from build123d import *

# Parameters (mm, degrees)
EXTRUDE_406_DEPTH   = 240
SKETCH_3_R          = 2.5
SKETCH_3_R_2        = 3
CUT_EXTRUDE_1_DEPTH = 10


with BuildPart() as part:
    # 草图1 → Extrude 406 (new body)
    with BuildSketch(Plane.XY):
        with BuildLine():
            Line((33, 50.785428571), (15, 50.785428571))
            Line((15, 50.785428571), (15, 50.285428571))
            Line((15, 50.285428571), (-15, 50.285428571))
            Line((-15, 50.285428571), (-15, 50.785428571))
            Line((-15, 50.785428571), (-33, 50.785428571))
            ThreePointArc((-33, 50.785428571), (-36.535533906, 49.320962477), (-38, 45.785428571))
            Line((-38, 45.785428571), (-38, 9.785428571))
            ThreePointArc((-38, 9.785428571), (-37.121320344, 7.664108228), (-35, 6.785428571))
            Line((-35, 6.785428571), (-25, 6.785428571))
            Line((-25, 6.785428571), (-25, 39.785428571))
            Line((-25, 39.785428571), (25, 39.785428571))
            Line((25, 39.785428571), (25, 6.785428571))
            Line((25, 6.785428571), (35, 6.785428571))
            ThreePointArc((35, 6.785428571), (37.121320344, 7.664108228), (38, 9.785428571))
            Line((38, 9.785428571), (38, 45.785428571))
            ThreePointArc((38, 45.785428571), (36.535533906, 49.320962477), (33, 50.785428571))
        make_face()
    extrude(amount=-EXTRUDE_406_DEPTH)

    # 草图3 → 切除-拉伸1 (cut)
    with BuildSketch(Plane(origin=(0, 50.785428571, 0), x_dir=(-1, 0, 0), z_dir=(0, 1, 0))):
        with Locations((-20, -24)):
            Circle(SKETCH_3_R)
        with Locations((20, -24)):
            Circle(SKETCH_3_R)
        with Locations((-20, -88)):
            Circle(SKETCH_3_R)
        with Locations((20, -88)):
            Circle(SKETCH_3_R)
        with Locations((-20, -152)):
            Circle(SKETCH_3_R)
        with Locations((20, -152)):
            Circle(SKETCH_3_R)
        with Locations((-20, -216)):
            Circle(SKETCH_3_R)
        with Locations((20, -216)):
            Circle(SKETCH_3_R)
        with Locations((-25, -73)):
            Circle(SKETCH_3_R_2)
        with Locations((25, -73)):
            Circle(SKETCH_3_R_2)
        with Locations((-25, -167)):
            Circle(SKETCH_3_R_2)
        with Locations((25, -167)):
            Circle(SKETCH_3_R_2)
    extrude(amount=-CUT_EXTRUDE_1_DEPTH, mode=Mode.SUBTRACT)


solid = part.part
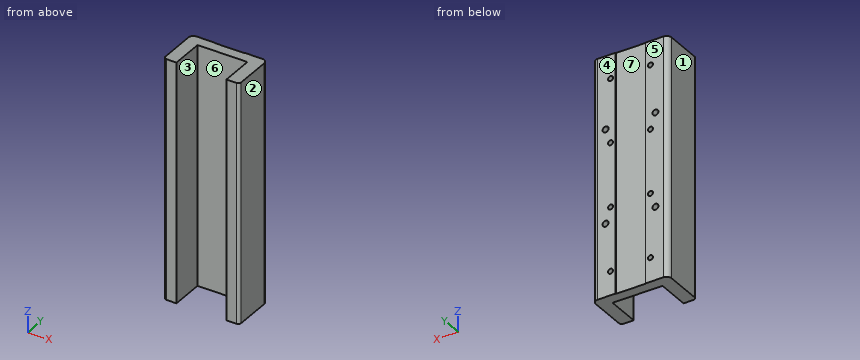
Part model, mm, in its own coordinate system. Face numbers are marked on the shaded views. A direction names the side the tool comes from. Coordinates: 2 decimals unless noted, no trailing zeros. Loops run counter-clockwise (first coordinate to the right, second up) from the corner with the lowest first, then second, coordinate; pieces in that order, holes last. Notation, with made-up numbers: (31.5, -34) - (76.5, -34) arc R15 ccw to (76.5, -23) - close; hole circle Ø3 at (3.5, 33). An arc over 180 degrees is marked (long way). Write each question's results on one line, items separated by ' | '. Start each with the question number.
Q1. Slice it at B-B on z = -73. Give the cut face in (x, y), and give its area (3 significant figures).
Q2. Which spindle directions (+Z, -Z, +X, -X, +Y, -Y) get a long thin tool onto all of the face, cutting with end or side? Do the marked faces 5, 6 and 7. Say none if no direction does.
Q3. Slice it at A-A on y = 31. Give the cut face in (x, z), and give its area (3 significant figures).
Q4. Probe line 1 along Z through (x, y) = (25, 45); line 2 along Z through (x, y) = (20, 47); line 3 along X through (y, z) = (45, -152). List the from-to ranges inside material, lowest first.
Q5. Drop flat-ended pins along their axis: pin 1 Ø1.8 at (x, z) = (-25.5, -167) entering from +Y; pin 2 Ø6.5 at (x, z) = (-20, -24) entering from +Y; pin 3 Ø12 at (x, z) = (13.5, -208) entering from -Y. Give the stop position or say it passes through.
Q6. Slice it at D-D on x = 7.5. Give the cut face in (y, z), and give its area (3 significant figures).
Q7. Slice it at C-C on y = 48. Give the number of separate pieces and of enclosed holes in the cut face, and give its area (3 significant figures).
Q8. Two-plate mould, pull along X, no slides. Class the marked faces 1, 2, 3 and 4: +X half, -X half, draft (parallel to the pull), parting line (faces both ways), or undercut.
Answer:
1) outline: (-38, 9.79) arc R3 ccw to (-35, 6.79) - (-25, 6.79) - (-25, 39.79) - (25, 39.79) - (25, 6.79) - (35, 6.79) arc R3 ccw to (38, 9.79) - (38, 45.79) arc R5 ccw to (33, 50.79) - (28, 50.79) - (28, 40.79) - (22, 40.79) - (22, 50.79) - (15, 50.79) - (15, 50.29) - (-15, 50.29) - (-15, 50.79) - (-22, 50.79) - (-22, 40.79) - (-28, 40.79) - (-28, 50.79) - (-33, 50.79) arc R5 ccw to (-38, 45.79) - close | area: 1,540 mm2
2) face 5: +Z, -Z, +X, -X, +Y | face 6: +Z, -Z, -Y | face 7: +Z, -Z, +Y
3) outline: (-38, -240) - (-25, -240) - (-25, 0) - (-38, 0) - close; (25, -240) - (38, -240) - (38, 0) - (25, 0) - close | area: 6,240 mm2
4) line 1: z = -240 to -170, -164 to -76, -70 to 0 | line 2: z = -240 to -218.5, -213.5 to -154.5, -149.5 to -90.5, -85.5 to -26.5, -21.5 to 0 | line 3: x = -38 to -22.5, -17.5 to 17.5, 22.5 to 38
5) pin 1: stops at y = 40.79 | pin 2: stops at y = 50.79 | pin 3: stops at y = 39.79
6) outline: (39.79, -240) - (50.29, -240) - (50.29, 0) - (39.79, 0) - close | area: 2,520 mm2
7) separate pieces: 1 | enclosed holes: 12 | area: 17,700 mm2
8) face 1: -X half | face 2: +X half | face 3: undercut | face 4: draft
